```python
from build123d import *

# Parameters (mm, degrees)
SKETCH_1_W                = 120
SKETCH_1_H                = 60
EXTRUDE_1_DEPTH           = 10
CHAMFER_1_SIZE            = 5
HOLE_WIZARD_M5_1_D        = 4.2
HOLE_WIZARD_M5_1_DEPTH    = 12.4
HOLE_WIZARD_M5_1_TIP      = 1.2618073
HOLE_WIZARD_1_D           = 6.6
HOLE_WIZARD_1_DEPTH       = 12.4
HOLE_WIZARD_1_CBORE_D     = 11
HOLE_WIZARD_1_CBORE_DEPTH = 6.8
HOLE_WIZARD_1_TIP         = 1.982840043
HOLE_WIZARD_2_D           = 5.5
HOLE_WIZARD_2_DEPTH       = 12.4
HOLE_WIZARD_2_CBORE_D     = 10
HOLE_WIZARD_2_CBORE_DEPTH = 5.7
HOLE_WIZARD_2_TIP         = 1.652366702


with BuildPart() as part:
    # 草图1 → 凸台-拉伸1 (new body)
    with BuildSketch(Plane(origin=(0, 0, 0), x_dir=(1, 0, 0), z_dir=(0, 1, 0))):
        Rectangle(SKETCH_1_W, SKETCH_1_H)
    extrude(amount=EXTRUDE_1_DEPTH)

    # 倒角1
    chamfer_1_edges = [part.edges().sort_by_distance(p)[0] for p in [
        (60, 5, 30),
        (-60, 5, 30),
        (-60, 5, -30),
        (60, 5, -30),
    ]]
    chamfer(chamfer_1_edges, length=CHAMFER_1_SIZE)

    # M5 螺纹孔1
    with Locations(Plane.XY.offset(30)):
        with Locations((-40, 5), (0, 5), (40, 5)):
            Hole(HOLE_WIZARD_M5_1_D / 2, depth=HOLE_WIZARD_M5_1_DEPTH)
            with Locations((0, 0, -(HOLE_WIZARD_M5_1_DEPTH + HOLE_WIZARD_M5_1_TIP / 2))):  # 118° drill point
                Cone(0, HOLE_WIZARD_M5_1_D / 2, HOLE_WIZARD_M5_1_TIP, mode=Mode.SUBTRACT)

    # 打孔尺寸(%根据)内六角圆柱头螺钉的类型1
    with Locations(Plane(origin=(0, 0, 0), x_dir=(-1, 0, 0), z_dir=(0, -1, 0))):
        with Locations((30, -15), (30, 15), (-30, -15), (-30, 15)):
            CounterBoreHole(HOLE_WIZARD_1_D / 2, HOLE_WIZARD_1_CBORE_D / 2, HOLE_WIZARD_1_CBORE_DEPTH, depth=HOLE_WIZARD_1_DEPTH)
            with Locations((0, 0, -(HOLE_WIZARD_1_DEPTH + HOLE_WIZARD_1_TIP / 2))):  # 118° drill point
                Cone(0, HOLE_WIZARD_1_D / 2, HOLE_WIZARD_1_TIP, mode=Mode.SUBTRACT)

    # 打孔尺寸(%根据)内六角圆柱头螺钉的类型2
    with Locations(Plane(origin=(0, 10, 0), x_dir=(1, 0, 0), z_dir=(0, 1, 0))):
        with Locations((0, -15), (0, 15)):
            CounterBoreHole(HOLE_WIZARD_2_D / 2, HOLE_WIZARD_2_CBORE_D / 2, HOLE_WIZARD_2_CBORE_DEPTH, depth=HOLE_WIZARD_2_DEPTH)
            with Locations((0, 0, -(HOLE_WIZARD_2_DEPTH + HOLE_WIZARD_2_TIP / 2))):  # 118° drill point
                Cone(0, HOLE_WIZARD_2_D / 2, HOLE_WIZARD_2_TIP, mode=Mode.SUBTRACT)


solid = part.part
```
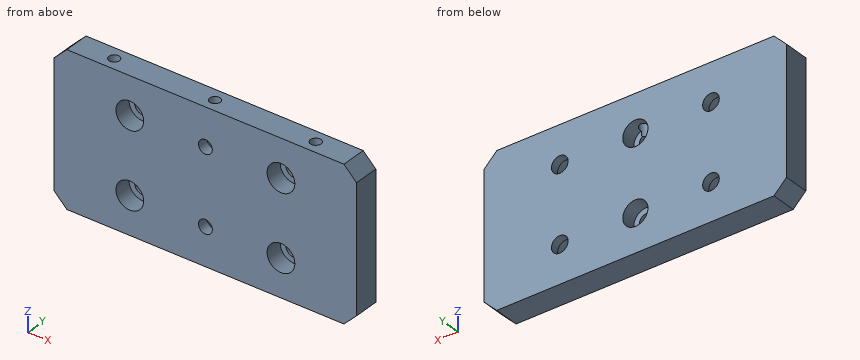
Model file for the job. Use its own axes, mm. Coordinates: 2 decimals unless noted, no trailing zeros. Order: outer loops, then holes, each group sorted by start corner. A loop starts at its lowest first (then second) coordinate and runs counter-clockwise, first axis right, second up. Notation, with made-up numbers: (-38, -6) - (-31, -6) arc R32 cw to (-31, 27) - close; hole circle Ø8 at (22, 18.25). An arc over 180 degrees is marked (long way). Return JSON: item names as keys, results as strings. Group by question number.
1) Saw through at B-B, the plane z = -16.5. Write the cut outline in (x, y), plus the area to 3 significant figures.
2) Flat gauge pins, fed straight in: P1, Ø4, axis at x = -30, z = -15, coming from the +Y side; P2, Ø2.5, axis at x = 40, y = 5, coming from the +Z side. Where does each tip first touch, or does it go through?
3) Saw through at A-A, the plane z = 15. Write the cut outline in (x, y), plus the area to 3 significant figures.
4) Probe line 1 (Z direction, x = -30, y = 8.1); line 2 (Z direction, x = -30, y = 5); line 3 (Y direction, x = 0, z = 20.5). List the from-to ranges inside material, lowest first. Write a range as from..to.
Values found:
{
 "1": {"outline": "(-60, 0) - (-35.29, 0) - (-35.29, 6.8) - (-32.94, 6.8) - (-32.94, 10) - (-60, 10) - close; (-27.06, 6.8) - (-24.71, 6.8) - (-24.71, 0) - (-2.3, 0) - (-2.3, 4.3) - (-4.77, 4.3) - (-4.77, 10) - (-27.06, 10) - close; (2.3, 0) - (24.71, 0) - (24.71, 6.8) - (27.06, 6.8) - (27.06, 10) - (4.77, 10) - (4.77, 4.3) - (2.3, 4.3) - close; (32.94, 6.8) - (35.29, 6.8) - (35.29, 0) - (60, 0) - (60, 10) - (32.94, 10) - close", "area": "944 mm²"},
 "2": {"P1": "passes through", "P2": "stops at z = 17.09"},
 "3": {"outline": "(-60, 0) - (-35.5, 0) - (-35.5, 6.8) - (-33.3, 6.8) - (-33.3, 10) - (-60, 10) - close; (-26.7, 6.8) - (-24.5, 6.8) - (-24.5, 0) - (-2.75, 0) - (-2.75, 4.3) - (-5, 4.3) - (-5, 10) - (-26.7, 10) - close; (2.75, 0) - (24.5, 0) - (24.5, 6.8) - (26.7, 6.8) - (26.7, 10) - (5, 10) - (5, 4.3) - (2.75, 4.3) - close; (33.3, 6.8) - (35.5, 6.8) - (35.5, 0) - (60, 0) - (60, 10) - (33.3, 10) - close", "area": "928 mm²"},
 "4": {"line 1": "z = -30..-18.3, -11.7..11.7, 18.3..30", "line 2": "z = -30..-20.5, -9.5..9.5, 20.5..30", "line 3": "y = 0..2.9, 7.1..10"}
}
